Read the model definition and answer for the solid it produces. Units are mm, in the model's axes. A direction names the side the tool comes from. Give positions to 0.01 mm unless a question says otherwise; leave off trailing zeros. Loops run counter-clockwise (first coordinate to the right, second up) from the corner with the lowest first, then second, coordinate; pieces in that order, holes last. Notation, with made-up numbers: (30, -4) - (51, -4) arc R13 ccw to (51, 1) - close; hole circle Ø1 at (34, -38.5). An arc over 180 degrees is marked (long way). Put each result on its own line as item: value. Start each with the question number.
1. A cutting plane is placed at C-C, the plane z = -17. Determine the outline of the cut face in (x, y).
2. Given pin 1 Ø7.5 at (x, z) = (16.5, 4.5) entering from +Y; pin 2 Ø8 at (y, z) = (18, -15.5) entering from +X, each flat-ended and moving along its own axis, determine where each tip first touches the part or whether it passes through.
3. A cutting plane is placed at A-A, the plane y = 28. Determine the outline of the cut face in (x, z).
4. Consider L1, parallel to Z at x = 2.5, y = 34.5; L2, parallel to X at y = 20, z = 7; L3, parallel to Y at x = 13.5, z = -1. Determine where each line is inside the solid, lowest interval first. Write a range as from..to.
5. A cutting plane is placed at B-B, the plane x = 5. Determine the outline of the cut face in (y, z).
6. For a pull along Z with two mould halves and no side action, classify faces 1 (the flat face through (6, 17, 20)), 2 (the flat face through (4, 37, 8.5)), 3 (the flat face through (23, 5, 0)) as released by +Z, released by -Z, zero draft, split by the parting line, or undercut.
7. A cutting plane is placed at D-D, the plane z = 0. Determine the outline of the cut face in (x, y), plus the area to 3 significant figures.
8. For faces 4 (the flat face through (6, 17, -20)), 5 (the flat face through (4, 37, -8.5)), 6 (the flat face through (8, 22, 0)), determine the directions among +Z, -Z, +X, -X, +Y, -Y from which every point of the face is accessible in a straight line to the end or side of a thin tool.
```python
from build123d import *

# Parameters (mm, degrees)
EXTRUDE_1_DEPTH     = 20
CUT_EXTRUDE_1_REACH = 50.877


with BuildPart() as part:
    # 草图1 → 凸台-拉伸1 (new, symmetric)
    with BuildSketch(Plane.XY):
        Polygon((0, 0), (23, 0), (23, 10), (8, 10), (8, 42), (0, 42), align=None)
    extrude(amount=EXTRUDE_1_DEPTH, both=True)

    # 草图2 → 切除-拉伸1 (cut, up to next)
    with BuildSketch(Plane(origin=(8, 0, 0), x_dir=(0, 0, -1), z_dir=(1, 0, 0)), mode=Mode.PRIVATE) as cut_extrude_1_sk1:
        with BuildLine():
            Line((-8.5, 42), (-8.5, 32))
            ThreePointArc((-8.5, 32), (0, 23.5), (8.5, 32))
            Line((8.5, 32), (8.5, 42))
            Line((8.5, 42), (-8.5, 42))
        make_face()
    cut_extrude_1_tool1 = extrude(cut_extrude_1_sk1.sketch, amount=-CUT_EXTRUDE_1_REACH, mode=Mode.PRIVATE) & part.part
    add(cut_extrude_1_tool1.solids().sort_by_distance((8, 33.55414, 0))[0], mode=Mode.SUBTRACT)


solid = part.part
```
Return value:
1. outline: (0, 0) - (23, 0) - (23, 10) - (8, 10) - (8, 42) - (0, 42) - close
2. pin 1: stops at y = 10
2. pin 2: stops at x = 8
3. outline: (0, -20) - (8, -20) - (8, -7.5) - (0, -7.5) - close; (0, 7.5) - (8, 7.5) - (8, 20) - (0, 20) - close
4. L1: z = -20..-8.5, 8.5..20
4. L2: x = 0..8
4. L3: y = 0..10
5. outline: (0, -20) - (42, -20) - (42, -8.5) - (32, -8.5) arc R8.5 cw to (32, 8.5) - (42, 8.5) - (42, 20) - (0, 20) - close
6. face 1: released by +Z
6. face 2: undercut
6. face 3: zero draft
7. outline: (0, 0) - (23, 0) - (23, 10) - (8, 10) - (8, 23.5) - (0, 23.5) - close
7. area: 338 mm2
8. face 4: -Z, +X, -X, +Y, -Y
8. face 5: +X, -X, +Y
8. face 6: +Z, -Z, +X, +Y
